```python
from build123d import *

# Parameters (mm, degrees)
SKETCH1_W           = 7
SKETCH1_H           = 4.8
BOSS_EXTRUDE1_DEPTH = 97
SKETCH2_R           = 1
CUT_EXTRUDE1_DEPTH  = 668
SKETCH3_R           = 2.5
CUT_EXTRUDE2_DEPTH  = 2.5
LPATTERN1_COUNT     = 7
LPATTERN1_PITCH     = 15


with BuildPart() as part:
    # Sketch1 → Boss-Extrude1 (new body)
    with BuildSketch(Plane.XY):
        with Locations((0, 0.250289017)):
            Rectangle(SKETCH1_W, SKETCH1_H)
    extrude(amount=BOSS_EXTRUDE1_DEPTH)

    # Sketch2 → Cut-Extrude1 (cut)
    with BuildSketch(Plane(origin=(0, 2.650289017, 0), x_dir=(1, 0, 0), z_dir=(0, 1, 0))):
        with Locations(Location((0, -92, 0), (0, 0, 270))):
            Circle(SKETCH2_R)
    cut_extrude1 = extrude(amount=-CUT_EXTRUDE1_DEPTH, mode=Mode.SUBTRACT)

    # Sketch3 → Cut-Extrude2 (cut)
    with BuildSketch(Plane(origin=(0, 2.650289017, 0), x_dir=(1, 0, 0), z_dir=(0, 1, 0))):
        with Locations(Location((0, -92, 0), (0, 0, 270))):
            Circle(SKETCH3_R)
    cut_extrude2 = extrude(amount=-CUT_EXTRUDE2_DEPTH, mode=Mode.SUBTRACT)

    # LPattern1: Cut-Extrude1, Cut-Extrude2 ×7
    with Locations(*[(0, 0, -i * LPATTERN1_PITCH) for i in range(1, LPATTERN1_COUNT)]):
        add(cut_extrude1, mode=Mode.SUBTRACT)
        add(cut_extrude2, mode=Mode.SUBTRACT)


solid = part.part
```
Geometry check sheet. Reference: the model listing, model coordinates, mm. A direction names the side the tool comes from. Coordinates: 2 decimals unless noted, no trailing zeros. Order: outer loops, then holes, each group sorted by start corner. A loop starts at its lowest first (then second) coordinate and runs counter-clockwise, first axis right, second up.
Item 1: Tool access check on faces 1 (the flat face through (-3.5, 0, 48)), 2 (the cylindrical face through (0.1, 1.4, 74.5)). Record the directions out of +Z, -Z, +X, -X, +Y, -Y that give a thin tool (end or side, any length) a straight path to the whole face; none if there is none.
Item 2: Section check C-C (x = 0). Count the separate pieces of the cut face and the enclosed holes in it, plus the area to 3 significant figures.
Item 3: Depth check by flat-ended pin: pin 1 (3 mm diameter, centred on x = 0, z = 47, fed in from -Y); pin 2 (1.2 mm diameter, centred on x = 0, z = 17, fed in from -Y); pin 3 (2.5 mm diameter, centred on x = 0, z = 47.5, fed in from +Y). Enter the tip coordinate at first touch or a pass-through.
Item 4: Mould release check, pull along X, two halves, no side actions. Record for faces 3 (the cylindrical face through (-1, -1, 2)), 4 (the flat face through (3.5, 0, 48)), 5 (the flat face through (-3, 2.65, 48)): released by +X, released by -X, zero draft, split by the parting line, or undercut.
Item 5: Section check B-B (y = 0.95). Enter the section's corners in (x, z), plus the area to 3 significant figures.
Item 6: Section check A-A (z = 17). Enter the section's corners in (x, y).
Item 7: Scan lines: line 1 along X through (y, z) = (-1.3, 62); line 2 along X through (y, z) = (1.3, 62); line 3 along Y through (x, z) = (1, 90). Record each from-to range of solid material in increasing order.
Check sheet entries:
1. face 1: +Z, -Z, -X, +Y, -Y
1. face 2: +Y
2. separate pieces: 8
2. enclosed holes: 0
2. area: 347 mm2
3. pin 1: stops at y = -2.15
3. pin 2: passes through
3. pin 3: stops at y = 0.15
4. face 3: undercut
4. face 4: released by +X
4. face 5: zero draft
5. outline: (-3.5, 0) - (-1.5, 0) arc R2.5 cw (long way) to (1.5, 0) - (3.5, 0) - (3.5, 97) - (-3.5, 97) - close; hole circle Ø5 at (0, 17); hole circle Ø5 at (0, 32); hole circle Ø5 at (0, 47); hole circle Ø5 at (0, 62); hole circle Ø5 at (0, 77); hole circle Ø5 at (0, 92)
5. area: 543 mm2
6. outline: (-3.5, -2.15) - (-1, -2.15) - (-1, 0.15) - (-2.5, 0.15) - (-2.5, 2.65) - (-3.5, 2.65) - close; (1, -2.15) - (3.5, -2.15) - (3.5, 2.65) - (2.5, 2.65) - (2.5, 0.15) - (1, 0.15) - close
7. line 1: x = -3.5 to -1, 1 to 3.5
7. line 2: x = -3.5 to -2.5, 2.5 to 3.5
7. line 3: y = -2.15 to 0.15
